```python
from build123d import *

# Parameters (mm, degrees)
SKETCH1_W           = 20
SKETCH1_H           = 30
SKETCH1_W_2         = 18
SKETCH1_H_2         = 28
BOSS_EXTRUDE1_DEPTH = 601
BOSS_EXTRUDE2_DEPTH = 1
SKETCH4_R           = 5
CUT_EXTRUDE1_DEPTH  = 633.095720599
SKETCH5_R           = 5
CUT_EXTRUDE2_DEPTH  = 633.061705848


with BuildPart() as part:
    # Sketch1 → Boss-Extrude1 (new body)
    with BuildSketch(Plane.XY):
        with Locations((10, -15)):
            Rectangle(SKETCH1_W, SKETCH1_H)
        with Locations((10, -15)):
            Rectangle(SKETCH1_W_2, SKETCH1_H_2, mode=Mode.SUBTRACT)
    extrude(amount=BOSS_EXTRUDE1_DEPTH)

    # Sketch3 → Boss-Extrude2 (add)
    with BuildSketch(Plane.ZY):
        with BuildLine():
            Line((571, -30), (601, -30))
            Line((601, -30), (628, -30))
            ThreePointArc((628, -30), (630.121320344, -29.121320344), (631, -27))
            Line((631, -27), (631, -3))
            ThreePointArc((631, -3), (630.121320344, -0.878679656), (628, 0))
            Line((628, 0), (601, 0))
            Line((601, 0), (571, 0))
            Line((571, 0), (571, -30))
        make_face()
    boss_extrude2 = extrude(amount=BOSS_EXTRUDE2_DEPTH)

    # Mirror2: Boss-Extrude2 across plane
    add(boss_extrude2.mirror(Plane(origin=(10, 0, 0), x_dir=(0, 0, 1), z_dir=(1, 0, 0))))

    # Sketch4 → Cut-Extrude1 (cut, through all)
    with BuildSketch(Plane(origin=(21, 0, 0), x_dir=(0, 0, -1), z_dir=(1, 0, 0))):
        with Locations(Location((-619.5, -15, 0), (0, 0, 90))):
            Circle(SKETCH4_R)
    extrude(amount=-CUT_EXTRUDE1_DEPTH, mode=Mode.SUBTRACT)

    # Sketch5 → Cut-Extrude2 (cut, through all)
    with BuildSketch(Plane.ZY):
        with Locations(Location((15, -15, 0), (0, 0, 270))):
            Circle(SKETCH5_R)
    extrude(amount=-CUT_EXTRUDE2_DEPTH, mode=Mode.SUBTRACT)


solid = part.part
```
Geometry check sheet. Reference: the model listing, model coordinates, mm. A direction names the side the tool comes from. Round coordinates to 2 decimals unless told otherwise and drop trailing zeros. Loops run counter-clockwise (first coordinate to the right, second up) from the corner with the lowest first, then second, coordinate; pieces in that order, holes last. Notation, with made-up numbers: (-34, 14.5) - (-3, 14.5) arc R20 cw to (-3, 43.5) - close; hole circle Ø3 at (63.25, -40). An arc over 180 degrees is marked (long way). Write item = value, one per line. Start each with the question number.
1. Section check C-C on z = 240.5. Enter the section's corners in (x, y).
2. Section check A-A on x = 12.25. Enter the section's corners in (y, z).
3. Mould release check, pull along Y, two halves, no side actions. Record for faces 5 (the face through (1, -15, 296)), 6 (the face through (10, 0, 318)), 7 (the face through (-1, -15, 601)), 8 (the face through (10, -30, 310)): released by +Y, released by -Y, zero draft, split by the parting line, or undercut.
4. Thickness scan on line 1 (Y direction, x = 20.7, z = 619.5); line 2 (X direction, y = -27, z = 384); line 3 (Y direction, x = 15.25, z = 122). Record the ranges inside material, lowest first.
5. Set-up check for faces 1 (the face through (20, -15, 612)), 2 (the face through (20, -15, 282)), 3 (the face through (10, -29, 296)), 4 (the face through (0, -15, 282)): record each of +Z, -Z, +X, -X, +Y, -Y from which the full face is reachable in a straight line by a thin tool's end or side.
6. Depth check by flat-ended pin: pin 1 (1 mm diameter, centred on y = -11.5, z = 404, fed in from -X); pin 2 (6 mm diameter, centred on x = 3.5, y = -7.5, fed in from +Z); pin 3 (11.5 mm diameter, centred on y = -15, z = 15, fed in from +X). Enter the tip coordinate at first touch or a pass-through.
7. Section check B-B on y = -15. Give the number of separate pieces and of enclosed holes in the cut face, then the cut area to 3 significant figures.
Working result:
q1.outline = (0, -30) - (20, -30) - (20, 0) - (0, 0) - close; hole (1, -29) - (19, -29) - (19, -1) - (1, -1) - close
q2.outline = (-30, 0) - (-29, 0) - (-29, 601) - (-30, 601) - close; (-1, 0) - (0, 0) - (0, 601) - (-1, 601) - close
q3.face_5 = undercut
q3.face_6 = released by +Y
q3.face_7 = zero draft
q3.face_8 = released by -Y
q4.line_1 = -30 to -20, -10 to 0
q4.line_2 = 0 to 1, 19 to 20
q4.line_3 = -30 to -29, -1 to 0
q5.face_1 = +Z, +Y, -Y
q5.face_2 = -Z, +X, +Y, -Y
q5.face_3 = +Z, -Z
q5.face_4 = -Z, -X, +Y, -Y
q6.pin_1 = 0
q6.pin_2 = 601
q6.pin_3 = 20
q7.separate_pieces = 6
q7.enclosed_holes = 0
q7.area = 1,280 mm^2
